The drawing under review shows one solid part. Ordinate dimensions are in mm from its lowest x, y, z. A direction names the side the tool comes from. Coordinates: 2 decimals unless noted, no trailing zeros. Write each loop counter-clockwise with the first axis right and the second up, starting at its lowest first coordinate (ties: lowest second). Pieces come first, ordered by that corner, then holes. Notation, with made-up numbers: (0.5, -31) -> (18.5, -31) arc R29 cw to (18.5, -10) -> close; hole circle Ø4 at (70.25, 61.25). An arc over 180 degrees is marked (long way). One line per question, with ' | ' between items. Start each with the question number.
Q1. Add section C-C on y = 28. State the section outline as (x, z) points, and give its area (3 significant figures).
Q2. For P1, Ø8, axis at x = 34, z = 18.5, coming from the +Y side; P2, Ø6, axis at x = 7, y = 33.5, coming from the +Z side; P3, Ø8, axis at x = 6, z = 16.5, coming from the +Y side, all flat-tipped, find the tip position at first contact; note any pin that passes through.
Q3. Add section D-D on z = 20.5. State the section outline as (x, y) points, and give its area (3 significant figures).
Q4. For the marked faces 1, 2 and 3, list the 3-axis set-ups (+Z, -Z, +X, -X, +Y, -Y) from which the entire face can be reached by the end or side of a thin tool; tool diameter is ignored.
Q5. Add section A-A on z = 16.5. State the section outline as (x, y) points.
Q6. Add section B-B on x = 20. State the section outline as (y, z) points.
Q7. Wall thickness on probe 1 along X at (y, z) = (5.65, 16.5); probe 2 along Z at (x, y) = (6, 5); probe 3 along Y at (x, z) = (20, 1.4): over which ranges is each line inside the solid? List them lowest first.
Q8. Draft analysis for pull direction X (two halves, no side actions). For the marked faces 4, 5 and 6, state which applies: pulls with the +X half, pulls with the -X half, needs draft (parallel to the pull), parting line crosses it, or undercut.
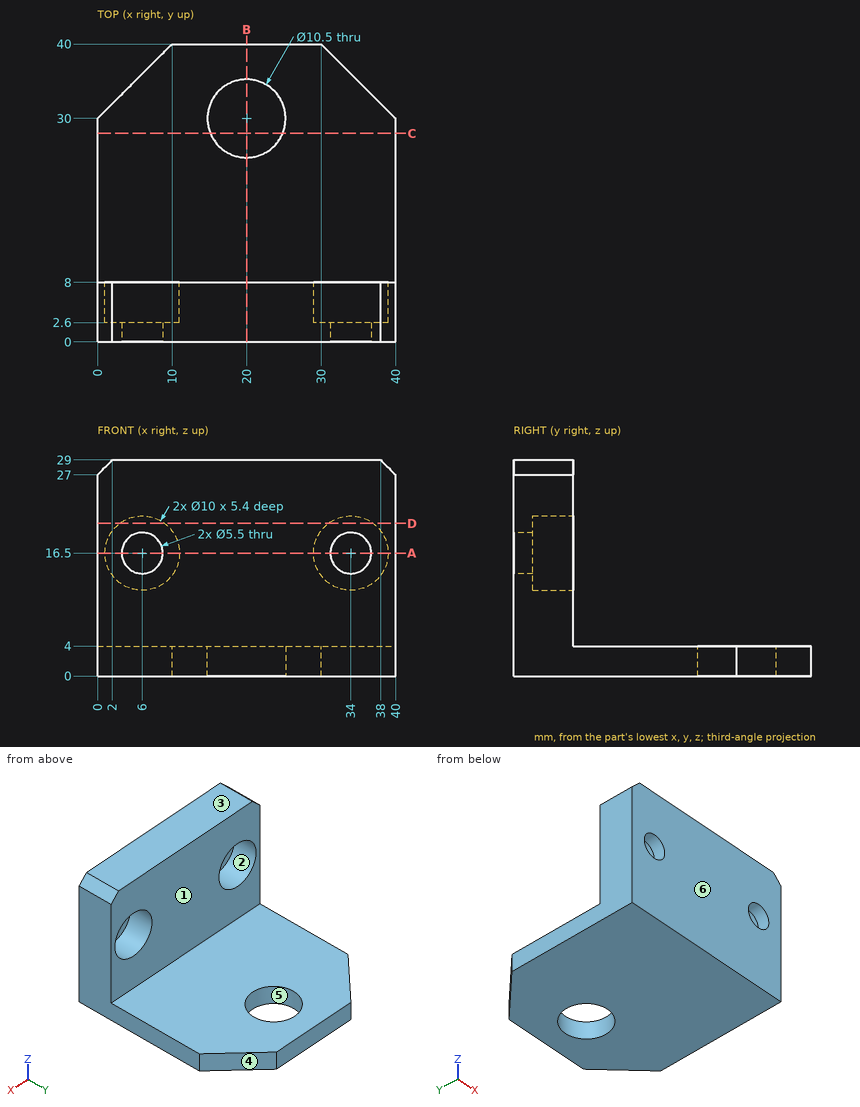
Output values:
1) outline: (0, 0) -> (15.15, 0) -> (15.15, 4) -> (0, 4) -> close; (24.85, 0) -> (40, 0) -> (40, 4) -> (24.85, 4) -> close | area: 121 mm2
2) P1: stops at y = 8 | P2: stops at z = 4 | P3: stops at y = 2.6
3) outline: (0, 0) -> (40, 0) -> (40, 8) -> (37, 8) -> (37, 2.6) -> (31, 2.6) -> (31, 8) -> (9, 8) -> (9, 2.6) -> (3, 2.6) -> (3, 8) -> (0, 8) -> close | area: 255 mm2
4) face 1: +Z, +X, -X, +Y | face 2: +Y | face 3: +Z, +X, -X, +Y, -Y
5) outline: (0, 0) -> (3.25, 0) -> (3.25, 2.6) -> (1, 2.6) -> (1, 8) -> (0, 8) -> close; (8.75, 0) -> (31.25, 0) -> (31.25, 2.6) -> (29, 2.6) -> (29, 8) -> (11, 8) -> (11, 2.6) -> (8.75, 2.6) -> close; (36.75, 0) -> (40, 0) -> (40, 8) -> (39, 8) -> (39, 2.6) -> (36.75, 2.6) -> close
6) outline: (0, 0) -> (24.75, 0) -> (24.75, 4) -> (8, 4) -> (8, 29) -> (0, 29) -> close; (35.25, 0) -> (40, 0) -> (40, 4) -> (35.25, 4) -> close
7) probe 1: x = 0 to 1, 11 to 29, 39 to 40 | probe 2: z = 0 to 11.5, 21.5 to 29 | probe 3: y = 0 to 24.75, 35.25 to 40
8) face 4: pulls with the +X half | face 5: undercut | face 6: needs draft
